Source: CAD feature listing. Evaluate the final solid. Frame: model axes, mm. Give positions to 0.01 mm unless a question says otherwise; leave off trailing zeros. Order: outer loops, then holes, each group sorted by start corner. A loop starts at its lowest first (then second) coordinate and runs counter-clockwise, first axis right, second up. Notation, with made-up numbers: M -25.75,20.25 L -13.75,20.25 A29 cw -13.75,45.25 Z; hole C 50.25,40 d2. An arc over 180 degrees is marked long. Return JSON: item names as keys, results as strings.
from build123d import *

# Parameters (mm, degrees)
SKETCH1_W                    = 16
SKETCH1_H                    = 70
EXTRUDE_THIN1_DEPTH          = 16
CHAMFER1_SIZE                = 1
SIZE_MM_BLIND_DOWEL_HOLE_1_D = 6
M8_TAPPED_HOLE1_D            = 6.8
M6_CLEARANCE_HOLE1_D         = 6.6


with BuildPart() as part:
    # Sketch1 → Extrude-Thin1 (new body)
    with BuildSketch(Plane.XY):
        with Locations((-8, 35)):
            Rectangle(SKETCH1_W, SKETCH1_H)
    extrude(amount=EXTRUDE_THIN1_DEPTH)

    # Chamfer1
    chamfer1_edges = [part.edges().sort_by_distance(p)[0] for p in [
        (-16, 70, 8),
        (0, 70, 8),
        (0, 0, 8),
        (-16, 0, 8),
    ]]
    chamfer(chamfer1_edges, length=CHAMFER1_SIZE)

    # Size mm blind dowel hole 1 (through all)
    with Locations(Plane.XY.offset(16)):
        with Locations((-8, 48), (-8, 22)):
            Hole(SIZE_MM_BLIND_DOWEL_HOLE_1_D / 2)

    # M8 Tapped Hole1 (through all)
    with Locations(Plane.ZY.offset(16)):
        with Locations((8, 35)):
            Hole(M8_TAPPED_HOLE1_D / 2)

    # M6 Clearance Hole1 (through all)
    with Locations(Plane.XY.offset(16)):
        with Locations((-8, 62), (-8, 8)):
            Hole(M6_CLEARANCE_HOLE1_D / 2)


solid = part.part
1. Section query A-A (x = -8). Return loops of the section in (y, z), then the cut area to 3 significant figures.
Evaluation:
{"outline": "M 0,0 L 4.7,0 L 4.7,16 L 0,16 Z; M 11.3,0 L 19,0 L 19,16 L 11.3,16 Z; M 25,0 L 45,0 L 45,16 L 25,16 Z; M 51,0 L 58.7,0 L 58.7,16 L 51,16 Z; M 65.3,0 L 70,0 L 70,16 L 65.3,16 Z; hole C 35,8 d6.8", "area": "680 mm^2"}
2. First-contact query: pin 1 (5.5 mm diameter, centred on x = -8, y = 62, fed in from +Z). Flat tip, straight axial feed; report the tip coordinate or a pass-through.
Evaluation:
{"pin 1": "passes through"}
3. Draft query along X for faces 1 (the face through (-8, 35, 16)), 2 (the face through (0, 35, 4)), 3 (the face through (-9.61, 50.53, 7.89)), 4 (the face through (-7.57, 65.27, 7.89)). Return one class per face: pulls with the +X half, pulls with the -X half, needs draft (parallel to the pull), parting line crosses it, or undercut.
Evaluation:
{"face 1": "needs draft", "face 2": "pulls with the +X half", "face 3": "undercut", "face 4": "undercut"}
4. Section query B-B (y = 8). Return loops of the section in (x, z), then the cut area to 3 significant figures.
Evaluation:
{"outline": "M -16,0 L -11.3,0 L -11.3,16 L -16,16 Z; M -4.7,0 L 0,0 L 0,16 L -4.7,16 Z", "area": "150 mm^2"}
5. Section query C-C (z = 14). Return loops of the section in (x, y), then the cut area to 3 significant figures.
Evaluation:
{"outline": "M -16,1 L -15,0 L -1,0 L 0,1 L 0,69 L -1,70 L -15,70 L -16,69 Z; hole C -8,8 d6.6; hole C -8,62 d6.6; hole C -8,22 d6; hole C -8,48 d6", "area": "993 mm^2"}
6. Section query D-D (z = 8). Return loops of the section in (x, y).
Evaluation:
{"outline": "M -16,1 L -15,0 L -1,0 L 0,1 L 0,31.6 L -16,31.6 Z; M -16,38.4 L 0,38.4 L 0,69 L -1,70 L -15,70 L -16,69 Z; hole C -8,8 d6.6; hole C -8,62 d6.6; hole C -8,22 d6; hole C -8,48 d6"}
7. Ray query, probe 1 along Y at (x, z) = (-5.25, 5.75); probe 2 along X at (y, z) = (64, 9.25); probe 3 along Z at (x, y) = (-4.75, 34). Return the intervals inside material, ascending.
Evaluation:
{"probe 1": "y = 0 to 6.18, 9.82 to 20.8, 23.2 to 32.45, 37.55 to 46.8, 49.2 to 60.18, 63.82 to 70", "probe 2": "x = -16 to -10.62, -5.38 to 0", "probe 3": "z = 0 to 4.75, 11.25 to 16"}
